Verification items for the finished model (mm, model axes). Coordinates: 2 decimals unless noted, no trailing zeros. Write each loop counter-clockwise with the first axis right and the second up, starting at its lowest first coordinate (ties: lowest second). Pieces come first, ordered by that corner, then holes. Notation, with made-up numbers: (10, 63.25) -> (32, 63.25) arc R22 cw to (32, 98.25) -> close; hole circle Ø6 at (88, 52.25). An arc over 180 degrees is marked (long way). Use CSV: the item, a comma, the result in double quotes.
```python
from build123d import *

# Parameters (mm, degrees)
SKETCH1_R           = 14
SKETCH1_R_2         = 8
BOSS_EXTRUDE1_DEPTH = 6
FILLET1_R           = 1
SKETCH2_R           = 4
CUT_EXTRUDE1_DEPTH  = 20


with BuildPart() as part:
    # Sketch1 → Boss-Extrude1 (new, symmetric)
    with BuildSketch(Plane.XY):
        Circle(SKETCH1_R)
        Circle(SKETCH1_R_2, mode=Mode.SUBTRACT)
    extrude(amount=BOSS_EXTRUDE1_DEPTH, both=True)

    # Fillet1
    fillet1_edges = [part.edges().sort_by_distance(p)[0] for p in [
        (-14, 0, -6),
        (-14, 0, 6),
    ]]
    fillet(fillet1_edges, radius=FILLET1_R)

    # Sketch2 → Cut-Extrude1 (cut)
    with BuildSketch(Plane(origin=(0, 0, 0), x_dir=(1, 0, 0), z_dir=(0, 1, 0))):
        with Locations(Location((0, 0, 0), (0, 0, 90))):
            Circle(SKETCH2_R)
    extrude(amount=CUT_EXTRUDE1_DEPTH, mode=Mode.SUBTRACT)


solid = part.part
```
1) Cross-section at C-C (z = -1.5). Record the boundary of the cut face in (x, y), plus the area to 3 significant figures.
Return value:
outline,"(-3.71, 7.09) -> (-3.71, 13.5) arc R14 ccw (long way) to (3.71, 13.5) -> (3.71, 7.09) arc R8 cw (long way) to start"
area,"369 mm2"
2) Cross-section at B-B (x = 0). Record the boundary of the cut face in (y, z), plus the area to 3 significant figures.
Return value:
outline,"(-14, -5) arc R1 ccw to (-13, -6) -> (-8, -6) -> (-8, 6) -> (-13, 6) arc R1 ccw to (-14, 5) -> close; (8, -6) -> (13, -6) arc R1 ccw to (14, -5) -> (14, -4) -> (8, -4) -> close; (8, 4) -> (14, 4) -> (14, 5) arc R1 ccw to (13, 6) -> (8, 6) -> close"
area,"95.1 mm2"
3) Cross-section at D-D (z = 0). Record the boundary of the cut face in (x, y).
Return value:
outline,"(-4, 6.93) -> (-4, 13.42) arc R14 ccw (long way) to (4, 13.42) -> (4, 6.93) arc R8 cw (long way) to start"
4) Gauge pin test, flat ends, axial feed: pin 1 (2 mm diameter, centred on y = 2, z = -4.5, fed in from +X); pin 2 (2 mm diameter, centred on y = -11, z = 3, fed in from +X); pin 3 (1 mm diameter, centred on y = -1.5, z = 0.5, fed in from -X); pin 4 (9.5 mm diameter, centred on x = 0, y = 0, fed in from +Z). Record the tip position at first contact, or that the pin passes through.
Return value:
pin 1,"x = 13.96"
pin 2,"x = 9.8"
pin 3,"x = -13.96"
pin 4,"through"
5) Cross-section at A-A (y = 0). Record the boundary of the cut face in (x, z), plus the area to 3 significant figures.
Return value:
outline,"(-14, -5) arc R1 ccw to (-13, -6) -> (-8, -6) -> (-8, 6) -> (-13, 6) arc R1 ccw to (-14, 5) -> close; (8, -6) -> (13, -6) arc R1 ccw to (14, -5) -> (14, 5) arc R1 ccw to (13, 6) -> (8, 6) -> close"
area,"143 mm2"
6) Mould release check, pull along X, two halves, no side actions. Record for faces 1 (the flat face through (6, 6, 6)), 2 (the cylindrical face through (-3.373, 10.415, -2.15)), 3 (the cylindrical face through (6.5, -12.4, 0.1)): released by +X, released by -X, zero draft, split by the parting line, or undercut.
Return value:
face 1,"zero draft"
face 2,"undercut"
face 3,"split by the parting line"
7) Scan lines: L1, parallel to Y at x = -2.5, z = 3.5; L2, parallel to Y at x = 0, z = 3; L3, parallel to Y at x = 4.25, z = -3.5. Record each from-to range of solid material in increasing order.
Return value:
L1,"-13.77 to -7.6, 7.6 to 13.77"
L2,"-14 to -8"
L3,"-13.34 to -6.78, 6.78 to 13.34"
